from build123d import *

# Parameters (mm, degrees)
BLOCK_PROFILE_62X50_W             = 62
BLOCK_PROFILE_62X50_H             = 50
BASE_BLOCK_62X50X50_DEPTH         = 50
SQUARE_CUT_A_PROFILE_34X34_R      = 17
SQUARE_CUT_A_34X34_DEPTH_12_DEPTH = 12
SIDE_ARC_CUT_A_DEPTH              = 95.042543564
SIDE_ARC_CUT_B_DEPTH_12_DEPTH     = 12
SQUARE_START                      = -12
SQUARE_CUT_B_PROFILE_34X34_R      = 17
SQUARE_CUT_B_34X34_DEPTH_12_DEPTH = 12
HOLE_PROFILE_20_R                 = 10
HOLE_20_DEPTH_12_DEPTH            = 12


with BuildPart() as part:
    # Block Profile 62x50 → Base Block 62x50x50 (new body)
    with BuildSketch(Plane.XY):
        with Locations((31, 25)):
            Rectangle(BLOCK_PROFILE_62X50_W, BLOCK_PROFILE_62X50_H)
    extrude(amount=BASE_BLOCK_62X50X50_DEPTH)

    # Square Cut A Profile 34x34 → Square Cut A 34x34 Depth 12 (cut)
    with BuildSketch(Plane.XY.offset(50)):
        with Locations((62, 25)):
            Circle(SQUARE_CUT_A_PROFILE_34X34_R)
        with Locations((0, 25)):
            Circle(SQUARE_CUT_A_PROFILE_34X34_R)
    extrude(amount=-SQUARE_CUT_A_34X34_DEPTH_12_DEPTH, mode=Mode.SUBTRACT)

    # Side Arc Cut A Profile → Side Arc Cut A (cut, through all)
    with BuildSketch(Plane.XY.offset(50)):
        Polygon((31, 42), (17, 42), (17, 50), (45, 50), (45, 42), align=None)
    extrude(amount=-SIDE_ARC_CUT_A_DEPTH, mode=Mode.SUBTRACT)

    # Side Arc Cut B Profile → Side Arc Cut B Depth 12 (cut)
    with BuildSketch(Plane.ZY):
        Polygon((25, 34), (19.475936602, 34), (19.475936602, 16), (32, 16), (32, 34), align=None)
    extrude(amount=-SIDE_ARC_CUT_B_DEPTH_12_DEPTH, mode=Mode.SUBTRACT)

    # Square Cut B Profile 34x34 → Square Cut B 34x34 Depth 12 (cut)
    with BuildSketch(Plane(origin=(0, 0, 0), x_dir=(-1, 0, 0), z_dir=(0, 0, -1)).offset(SQUARE_START)):
        with Locations((-62, 25)):
            Circle(SQUARE_CUT_B_PROFILE_34X34_R)
        with Locations((0, 25)):
            Circle(SQUARE_CUT_B_PROFILE_34X34_R)
    extrude(amount=SQUARE_CUT_B_34X34_DEPTH_12_DEPTH, mode=Mode.SUBTRACT)

    # Hole Profile Ø20 → Hole Ø20 Depth 12 (cut)
    with BuildSketch(Plane.XY.offset(50)):
        with Locations((31, 25)):
            Circle(HOLE_PROFILE_20_R)
    extrude(amount=-HOLE_20_DEPTH_12_DEPTH, mode=Mode.SUBTRACT)


solid = part.part
The model under review builds one solid part; all positions refer to its coordinate system, in mm. A direction names the side the tool comes from. Give positions to 0.01 mm unless a question says otherwise; leave off trailing zeros. Order: outer loops, then holes, each group sorted by start corner. A loop starts at its lowest first (then second) coordinate and runs counter-clockwise, first axis right, second up. Notation, with made-up numbers: M 5,-1 L 53,-1 A29 cw 53,30 Z; hole C 71.5,35.25 d1. An arc over 180 degrees is marked long. Use one line per item in the form item = value. Start each with the question number.
Item 1: Insertion check: pin 1 Ø9.5 at (x, y) = (3.5, 29.5) entering from -Z; pin 2 Ø8.5 at (x, z) = (33, 23) entering from +Y; pin 3 Ø5 at (x, y) = (10, 31) entering from +Z. Each pin has a flat end and moves straight along its axis. Give the tip position at first contact, or say it passes through.
Item 2: We need section B-B on y = 25. Give the boundary of the cut face in (x, z).
Item 3: To check wall thickness, follow line 1 along Y through (x, z) = (31, 46); line 2 along Y through (x, z) = (19, 33); line 3 along Z through (x, y) = (8, 29). State the ranges of each line that lie inside material, in increasing order. Write a range as from..to.
Item 4: For faces 1 (the flat face through (6, 16, 26)), 2 (the cylindrical face through (17, 25, 44)), 3 (the cylindrical face through (45, 25, 6)), 4 (the cylindrical face through (40.54, 28, 44.08)), list the 3-axis set-ups (+Z, -Z, +X, -X, +Y, -Y) from which the entire face can be reached by the end or side of a thin tool; tool diameter is ignored.
Item 5: The part is to be moulded in two halves that separate along Y. For faces 5 (the flat face through (31, 25, 0)), 6 (the flat face through (31, 25, 38)), 7 (the flat face through (53, 50, 25)), say which applies: pulls with the +Y half, pulls with the -Y half, needs draft (parallel to the pull), parting line crosses it, or undercut.
Item 6: We need section C-C on z = 6. Give the boundary of the cut face in (x, y), plus the area to 3 significant figures.
Item 7: We need section D-D on x = 7. Give the boundary of the cut face in (y, z).
Item 8: We need section A-A on x = 31. Give the boundary of the cut face in (y, z).
Completed:
q1.pin_1 = 12
q1.pin_2 = 42
q1.pin_3 = 38
q2.outline = M 0,12 L 17,12 L 17,0 L 45,0 L 45,12 L 62,12 L 62,38 L 45,38 L 45,50 L 41,50 L 41,38 L 21,38 L 21,50 L 17,50 L 17,38 L 0,38 L 0,32 L 12,32 L 12,19.48 L 0,19.48 Z
q3.line_1 = 0..15, 35..42
q3.line_2 = 0..42
q3.line_3 = 12..19.48, 32..38
q4.face_1 = -X
q4.face_2 = +Z, -X
q4.face_3 = -Z, +X
q4.face_4 = +Z
q5.face_5 = needs draft
q5.face_6 = undercut
q5.face_7 = pulls with the +Y half
q6.outline = M 0,0 L 62,0 L 62,8 A17 cw 62,42 L 62,50 L 45,50 L 45,42 L 17,42 L 17,50 L 0,50 L 0,42 A17 cw 0,8 Z
q6.area = 1,970 mm²
q7.outline = M 0,0 L 9.51,0 L 9.51,12 L 40.49,12 L 40.49,0 L 50,0 L 50,50 L 40.49,50 L 40.49,38 L 9.51,38 L 9.51,50 L 0,50 Z; hole M 16,19.48 L 34,19.48 L 34,32 L 16,32 Z
q8.outline = M 0,0 L 42,0 L 42,50 L 35,50 L 35,38 L 15,38 L 15,50 L 0,50 Z
